Geometry: see drawing. Coordinates: mm, zero at the bounding-box minimum. Round coordinates to 2 decimals unless told otherwise and drop trailing zeros. Loops run counter-clockwise (first coordinate to the right, second up) from the corner with the lowest first, then second, coordinate; pieces in that order, holes last.
(1) First-contact query: pin 1 Ø12 at (y, z) = (108.5, 99) entering from -X; pin 2 Ø10 at (y, z) = (19.5, 202.5) entering from -X; pin 3 Ø1 at (y, z) = (21.5, 32) entering from +X. Flat tips, straight axial feed; report the tip coordinate or a pass-through.
(2) Mould query, pull axis Z, two halves, no side actions, for the marked faces 1 and 2. Classes: pulls with the +Z half, pulls with the -Z half, needs draft (parallel to the pull), parting line crosses it, or undercut.
(3) Section C-C, the plane y = 123. Return the cut outline in (x, z), plus the area to 3 significant figures.
(4) Section A-A, the plane z = 109.5. Return the cut outline in (x, y), plus the area to 3 significant figures.
(5) Section B-B, the plane x = 109.5. Return the cut outline in (y, z), plus the area to 3 significant figures.
(6) Section D-D, the plane y = 10.5. Return the cut outline in (x, z), plus the area to 3 significant figures.
(7) Material intervals for probe 1 along X at (y, z) = (67, 109); probe 2 along X at (y, z) = (24.5, 85.5); probe 3 along Z at (x, y) = (178.5, 47) (3 decimals), sorted ascending.
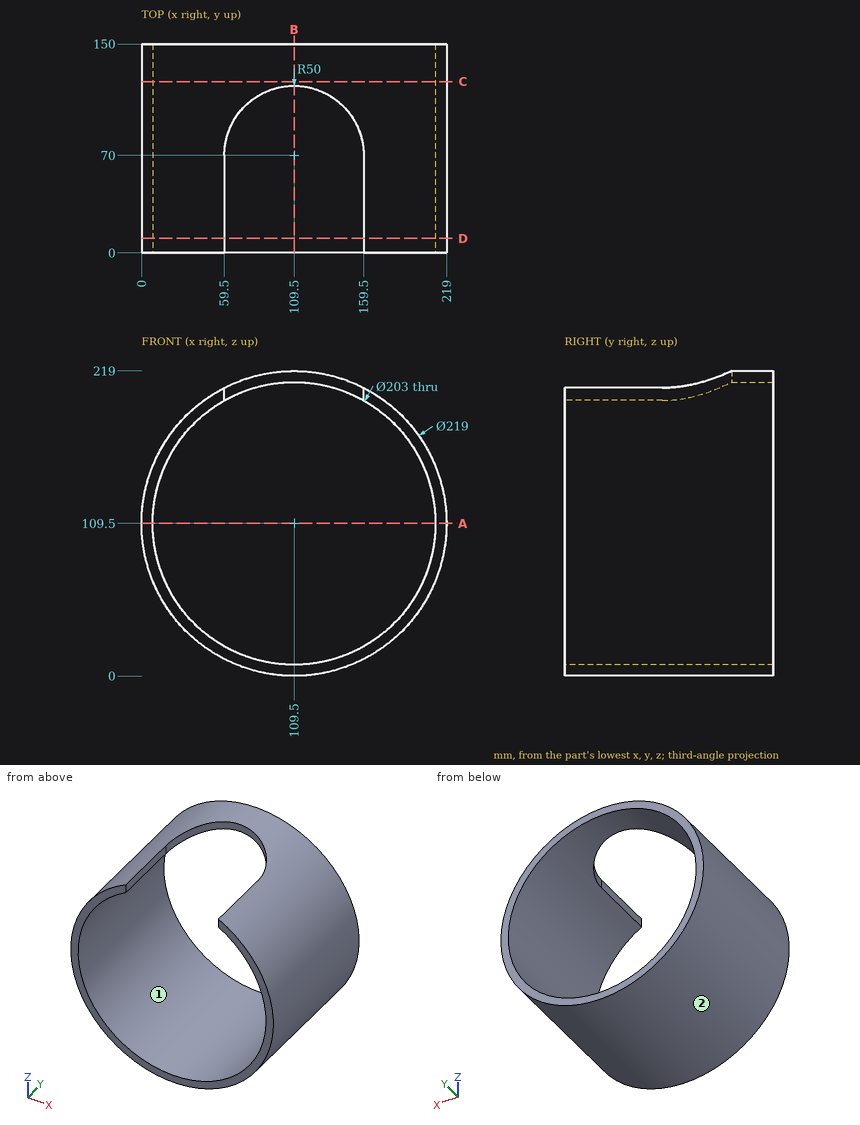
Output values:
1. pin 1: stops at x = 0.09
1. pin 2: stops at x = 44.34
1. pin 3: stops at x = 187.35
2. face 1: undercut
2. face 2: parting line crosses it
3. outline: circle Ø219 at (109.5, 109.5); hole circle Ø203 at (109.5, 109.5)
3. area: 5,300 mm2
4. outline: (0, 0) - (8, 0) - (8, 150) - (0, 150) - close; (211, 0) - (219, 0) - (219, 150) - (211, 150) - close
4. area: 2,400 mm2
5. outline: (0, 0) - (150, 0) - (150, 8) - (0, 8) - close; (120, 211) - (150, 211) - (150, 219) - (120, 219) - close
5. area: 1,440 mm2
6. outline: (59.5, 197.83) - (59.5, 206.92) arc R109.5 ccw (long way) to (159.5, 206.92) - (159.5, 197.83) arc R101.5 cw (long way) to start
6. area: 4,470 mm2
7. probe 1: x = 0 to 8, 211 to 219
7. probe 2: x = 2.66 to 10.88, 208.12 to 216.34
7. probe 3: z = 24.475 to 35.06, 183.94 to 194.525
